CAD build for the part. Positions are in the model's coordinates, mm. Round coordinates to 2 decimals unless told otherwise and drop trailing zeros. Order: outer loops, then holes, each group sorted by start corner. A loop starts at its lowest first (then second) coordinate and runs counter-clockwise, first axis right, second up. Notation, with made-up numbers: (28, 64.5) - (46, 64.5) arc R15 ccw to (46, 93.5) - close; hole circle Ø7 at (-25.5, 4.25). An arc over 180 degrees is marked (long way). Use one line per item in the form item = value. Start each with the question number.
from build123d import *

# Parameters (mm, degrees)
SKETCH1_W                                           = 150
SKETCH1_H                                           = 40
BOSS_EXTRUDE1_DEPTH                                 = 10
SKETCH2_R                                           = 4.75
CUT_EXTRUDE1_DEPTH                                  = 79.262379212
F_10_5_10_5_DIAMETER_HOLE1_D                        = 10.5
F_10_5_10_5_DIAMETER_HOLE1_DEPTH                    = 76
F_10_5_10_5_DIAMETER_HOLE1_TIP                      = 3.15451825
CBORE_FOR_M5_HEX_SOCKET_HEAD_CAP_SCREW1_D           = 5.5
CBORE_FOR_M5_HEX_SOCKET_HEAD_CAP_SCREW1_CBORE_D     = 10
CBORE_FOR_M5_HEX_SOCKET_HEAD_CAP_SCREW1_CBORE_DEPTH = 5.4
M4_TAPPED_HOLE1_REACH                               = 87.586
M4_TAPPED_HOLE1_BORE_R                              = 1.65
CHAMFER1_SIZE                                       = 3


with BuildPart() as part:
    # Sketch1 → Boss-Extrude1 (new body)
    with BuildSketch(Plane.XY):
        Rectangle(SKETCH1_W, SKETCH1_H)
    extrude(amount=BOSS_EXTRUDE1_DEPTH)

    # Sketch2 → Cut-Extrude1 (cut, through all)
    with BuildSketch(Plane.XY.offset(10)):
        with Locations((40, 2)):
            Circle(SKETCH2_R)
    extrude(amount=-CUT_EXTRUDE1_DEPTH, mode=Mode.SUBTRACT)

    # Ø10.5 (10.5) Diameter Hole1
    with Locations(Plane.XY.offset(10)):
        with Locations((0, 2)):
            Hole(F_10_5_10_5_DIAMETER_HOLE1_D / 2, depth=F_10_5_10_5_DIAMETER_HOLE1_DEPTH)
            with Locations((0, 0, -(F_10_5_10_5_DIAMETER_HOLE1_DEPTH + F_10_5_10_5_DIAMETER_HOLE1_TIP / 2))):  # 118° drill point
                Cone(0, F_10_5_10_5_DIAMETER_HOLE1_D / 2, F_10_5_10_5_DIAMETER_HOLE1_TIP, mode=Mode.SUBTRACT)

    # CBORE for M5 Hex Socket Head Cap Screw1 (through all)
    with Locations(Plane.XY.offset(10)):
        with Locations((60, 14), (0, 14), (-60, 14)):
            CounterBoreHole(CBORE_FOR_M5_HEX_SOCKET_HEAD_CAP_SCREW1_D / 2, CBORE_FOR_M5_HEX_SOCKET_HEAD_CAP_SCREW1_CBORE_D / 2, CBORE_FOR_M5_HEX_SOCKET_HEAD_CAP_SCREW1_CBORE_DEPTH)

    # M4 Tapped Hole1 bore → M4 Tapped Hole1 (cut, up to next)
    with BuildSketch(Plane(origin=(0, 20, 0), x_dir=(1, 0, 0), z_dir=(0, 1, 0)), mode=Mode.PRIVATE) as m4_tapped_hole1_sk1:
        with Locations((40, -5)):
            Circle(M4_TAPPED_HOLE1_BORE_R)
    m4_tapped_hole1_tool1 = extrude(m4_tapped_hole1_sk1.sketch, amount=-M4_TAPPED_HOLE1_REACH, mode=Mode.PRIVATE) & part.part
    add(m4_tapped_hole1_tool1.solids().sort_by_distance((40, 20, 5))[0], mode=Mode.SUBTRACT)

    # Chamfer1
    chamfer1_edges = [part.edges().sort_by_distance(p)[0] for p in [
        (75, -20, 5),
        (-75, -20, 5),
        (-75, 20, 5),
        (75, 20, 5),
    ]]
    chamfer(chamfer1_edges, length=CHAMFER1_SIZE)


solid = part.part
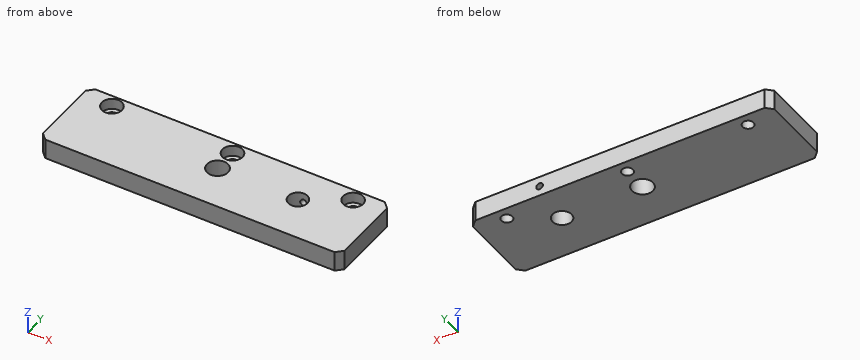
(1) Slice it at B-B (x = 40). Give the cut face in (y, z).
(2) Slice it at C-C (y = 2). Give the cut face in (x, z).
(3) Flat gauge pins, fed straight in: P1, Ø5, axis at x = 1.5, y = 15.5, coming from the +Z side; P2, Ø6.5, axis at x = 0, y = 2, coming from the +Z side; P3, Ø2, axis at x = 40, z = 5, coming from the +Y side. Where does each tip first touch, or does it go through?
(4) Slice it at A-A (y = 14). Give the number of separate pieces and of enclosed holes in the cut face, and give its area (3 significant figures).
(5) Wall check: line 1 (Y direction, x = 0, z = 8.1); line 2 (X direction, y = 3, z = 7); line 3 (X direction, y = 1.5, z = 5.25). Give the ranges that are in metal, low to high. Write a range as [from, to].
Results list:
q1.outline = (-20, 0) - (-2.75, 0) - (-2.75, 10) - (-20, 10) - close; (6.75, 0) - (20, 0) - (20, 3.35) - (6.75, 3.35) - close; (6.75, 6.65) - (20, 6.65) - (20, 10) - (6.75, 10) - close
q2.outline = (-75, 0) - (-5.25, 0) - (-5.25, 10) - (-75, 10) - close; (5.25, 0) - (35.25, 0) - (35.25, 10) - (5.25, 10) - close; (44.75, 0) - (75, 0) - (75, 10) - (44.75, 10) - close
q3.P1 = 4.6
q3.P2 = through
q3.P3 = -2.64
q4.separate_pieces = 4
q4.enclosed_holes = 1
q4.area = 1,250 mm²
q5.line_1 = [-20, -3.25], [7.25, 9], [19, 20]
q5.line_2 = [-75, -5.15], [5.15, 35.36], [44.64, 75]
q5.line_3 = [-75, -5.23], [5.23, 35.28], [44.72, 75]
